Work out the finished part from the listing and answer in its coordinate system (mm). A direction names the side the tool comes from. Coordinates: 2 decimals unless noted, no trailing zeros. Loops run counter-clockwise (first coordinate to the right, second up) from the corner with the lowest first, then second, coordinate; pieces in that order, holes last. Notation, with made-up numbers: (49, -37.75) -> (105, -37.75) arc R28 ccw to (105, 1.25) -> close; hole circle Ø5 at (69.5, -2). An arc over 180 degrees is marked (long way). Answer as CSV lines item,"result".
```python
from build123d import *

# Parameters (mm, degrees)
SKETCH_1_W          = 400
SKETCH_1_H          = 800
EXTRUDE_1_DEPTH     = 30
SHELL_1_T           = -2
SKETCH_2_W          = 35
SKETCH_2_H          = 120
CUT_EXTRUDE_1_DEPTH = 28
SKETCH_3_W          = 400
SKETCH_3_H          = 800
EXTRUDE_2_DEPTH     = 2


with BuildPart() as part:
    # 草图1 → 凸台-拉伸1 (new body)
    with BuildSketch(Plane(origin=(0, 0, 0), x_dir=(1, 0, 0), z_dir=(0, 1, 0))):
        with Locations((200, 400)):
            Rectangle(SKETCH_1_W, SKETCH_1_H)
    extrude(amount=EXTRUDE_1_DEPTH)

    # 抽壳1
    shell_1_openings = [part.faces().sort_by_distance(p)[0] for p in [
        (200, 30, -400),
    ]]
    offset(amount=SHELL_1_T, openings=shell_1_openings, kind=Kind.INTERSECTION)

    # 草图2 → 切除-拉伸1 (cut)
    with BuildSketch(Plane.XZ):
        with Locations((52.5, -460)):
            Rectangle(SKETCH_2_W, SKETCH_2_H)
    extrude(amount=-CUT_EXTRUDE_1_DEPTH, mode=Mode.SUBTRACT)

    # 草图3 → 凸台-拉伸2 (add)
    with BuildSketch(Plane(origin=(0, 30, 0), x_dir=(1, 0, 0), z_dir=(0, 1, 0))):
        with Locations((200, 400)):
            Rectangle(SKETCH_3_W, SKETCH_3_H)
    extrude(amount=-EXTRUDE_2_DEPTH)


solid = part.part
```
(1) A cutting plane is placed at A-A, the plane x = 104. Write down the section's boundary in (y, z).
Computed values:
outline,"(0, -800) -> (30, -800) -> (30, 0) -> (0, 0) -> close; hole (2, -798) -> (28, -798) -> (28, -2) -> (2, -2) -> close"
(2) For a pull along X with two mould halves and no side action, classify faces 3 (the face through (197, 30, -406)), 4 (the face through (398, 15, -394)), 5 (the face through (400, 15, -394)), 6 (the face through (197, 15, -798)) as pulls with the +X half, pulls with the -X half, needs draft (parallel to the pull), parting line crosses it, or undercut.
Computed values:
face 3,"needs draft"
face 4,"undercut"
face 5,"pulls with the +X half"
face 6,"undercut"
(3) A flat-ended cylindrical pin translates along its axis: pin 1 Ø10 at (x, z) = (292.5, -85) entering from -Y. Find the tip coordinate at first contact, or state that the pin passes through.
Computed values:
pin 1,"y = 0"
(4) Which of the six approach directions +Z, -Z, +X, -X, +Y, -Y give full straight-line access (tool end or side, diameter ignored) to faces 1 (the face through (197, 2, -406)), 2 (the face through (197, 15, -800))?
Computed values:
face 1,"none"
face 2,"-Z, +X, -X, +Y, -Y"
(5) A cutting plane is placed at B-B, the plane z = -368. Write down the section's boundary in (x, y).
Computed values:
outline,"(0, 0) -> (400, 0) -> (400, 30) -> (0, 30) -> close; hole (2, 2) -> (398, 2) -> (398, 28) -> (2, 28) -> close"
(6) Consider line 1 along Y through (x, z) = (243, -105); line 2 along X through (y, z) = (25.75, -728.5); line 3 along Z through (x, y) = (109.5, 5.25). Determine where each line is inside the solid, lowest interval first.
Computed values:
line 1,"0 to 2, 28 to 30"
line 2,"0 to 2, 398 to 400"
line 3,"-800 to -798, -2 to 0"
(7) A cutting plane is placed at C-C, the plane z = -502. Write down the section's boundary in (x, y).
Computed values:
outline,"(0, 0) -> (35, 0) -> (35, 2) -> (2, 2) -> (2, 28) -> (398, 28) -> (398, 2) -> (70, 2) -> (70, 0) -> (400, 0) -> (400, 30) -> (0, 30) -> close"
